from build123d import *

# Parameters (mm, degrees)
SKETCH_1_W               = 1210
SKETCH_1_H               = 210
EXTRUDE_1_DEPTH          = 30
SHELL_1_T                = -2
SKETCH_2_W               = 1210
SKETCH_2_H               = 20
EXTRUDE_2_DEPTH          = 2
SKETCH_3_R               = 4.5
CUT_EXTRUDE_1_DEPTH      = 94
CUT_EXTRUDE_2_DEPTH      = 1515
CUT_EXTRUDE_2_DEPTH_BACK = 94
SKETCH_4_R               = 4.5


with BuildPart() as part:
    # 草图1 → 凸台-拉伸1 (new body)
    with BuildSketch(Plane.XY):
        with Locations((605, 105)):
            Rectangle(SKETCH_1_W, SKETCH_1_H)
    extrude(amount=EXTRUDE_1_DEPTH)

    # 抽壳1
    shell_1_openings = [part.faces().sort_by_distance(p)[0] for p in [
        (605, 105, 30),
    ]]
    offset(amount=SHELL_1_T, openings=shell_1_openings, kind=Kind.INTERSECTION)

    # 草图2 → 凸台-拉伸2 (add)
    with BuildSketch(Plane.XY.offset(30)):
        with Locations((605, 220)):
            Rectangle(SKETCH_2_W, SKETCH_2_H)
    extrude(amount=-EXTRUDE_2_DEPTH)

    # 草图3 → 切除-拉伸1 (cut)
    with BuildSketch(Plane(origin=(0, 2, 0), x_dir=(1, 0, 0), z_dir=(0, 1, 0))):
        with Locations(Location((30, -16, 0), (0, 0, 270))):
            Circle(SKETCH_3_R)
        with Locations(Location((1180, -16, 0), (0, 0, 270))):
            Circle(SKETCH_3_R)
        with Locations(Location((605, -16, 0), (0, 0, 270))):
            Circle(SKETCH_3_R)
    extrude(amount=-CUT_EXTRUDE_1_DEPTH, mode=Mode.SUBTRACT)

    # 草图4 → 切除-拉伸2 (cut, two sides: drawn at the far end of the back side and taken through both)
    with BuildSketch(Plane(origin=(2, 0, 0), x_dir=(0, 0, -1), z_dir=(1, 0, 0)).offset(-CUT_EXTRUDE_2_DEPTH_BACK)):
        with Locations(Location((-16, 180, 0), (0, 0, 180))):
            Circle(SKETCH_4_R)
        with Locations(Location((-16, 30, 0), (0, 0, 180))):
            Circle(SKETCH_4_R)
    extrude(amount=CUT_EXTRUDE_2_DEPTH + CUT_EXTRUDE_2_DEPTH_BACK, mode=Mode.SUBTRACT)


solid = part.part
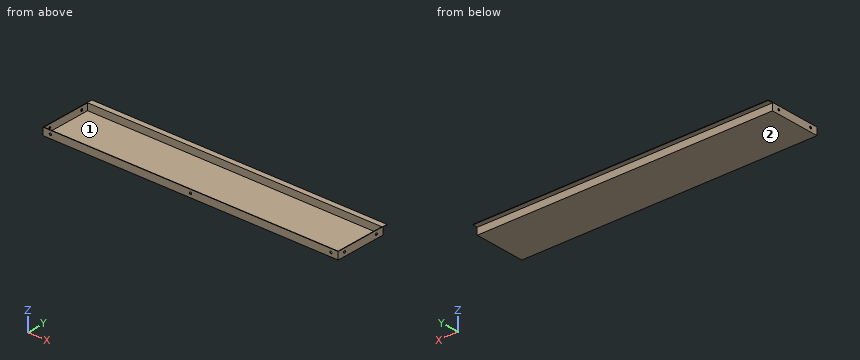
Check sheet for the modelled part. Datum: model origin and axes. Units: mm. Face numbers are marked on the shaded views. Give positions to 0.01 mm unless a question says otherwise; leave off trailing zeros. Write each loop counter-clockwise with the first axis right and the second up, starting at its lowest first coordinate (ties: lowest second). Pieces come first, ordered by that corner, then holes. Notation, with made-up numbers: M 63.25,71 L 112.25,71 A17 cw 112.25,101 Z; hole C 83,88 d5. An arc over 180 degrees is marked long. Use one line per item in the form item = value.
(1) Depth check by flat-ended pin: P1, Ø5.5, axis at x = 30, z = 16, coming from the -Y side; P2, Ø4, axis at x = 981, z = 13.5, coming from the -Y side; P3, Ø14, axis at x = 604.5, z = 17, coming from the +Y side; P4, Ø7, axis at y = 180, z = 16, coming from the +X side. Enter the tip coordinate at first touch or a pass-through.
Answer block:
P1 = 208
P2 = 0
P3 = 210
P4 = through
(2) Draft check along Y on the marked faces 1 and 2. Enter one of: pulls with the +Y half, pulls with the -Y half, needs draft (parallel to the pull), parting line crosses it, or undercut.
Answer block:
face_1 = undercut
face_2 = needs draft
(3) Material ranges on line 1 along X through (y, z) = (1.55, 16); line 2 along Y through (x, z) = (1209.55, 16); line 3 along Y through (x, z) = (224, 22.75), recorded low to high.
Answer block:
line_1 = 0 to 25.5, 34.5 to 600.5, 609.5 to 1175.5, 1184.5 to 1210
line_2 = 0 to 25.5, 34.5 to 175.5, 184.5 to 210
line_3 = 0 to 2, 208 to 210
(4) Section check C-C on z = 16. State how many separate pieces and enclosed holes the cut face has, plus the area to 3 significant figures.
Answer block:
separate_pieces = 7
enclosed_holes = 0
area = 5,540 mm2
(5) Section check A-A on y = 72. Record the boundary of the cut face in (x, z).
Answer block:
outline = M 0,0 L 1210,0 L 1210,30 L 1208,30 L 1208,2 L 2,2 L 2,30 L 0,30 Z
(6) Section check B-B on x = 940. Record the boundary of the cut face in (y, z), plus the area to 3 significant figures.
Answer block:
outline = M 0,0 L 210,0 L 210,28 L 230,28 L 230,30 L 208,30 L 208,2 L 2,2 L 2,30 L 0,30 Z
area = 572 mm2
